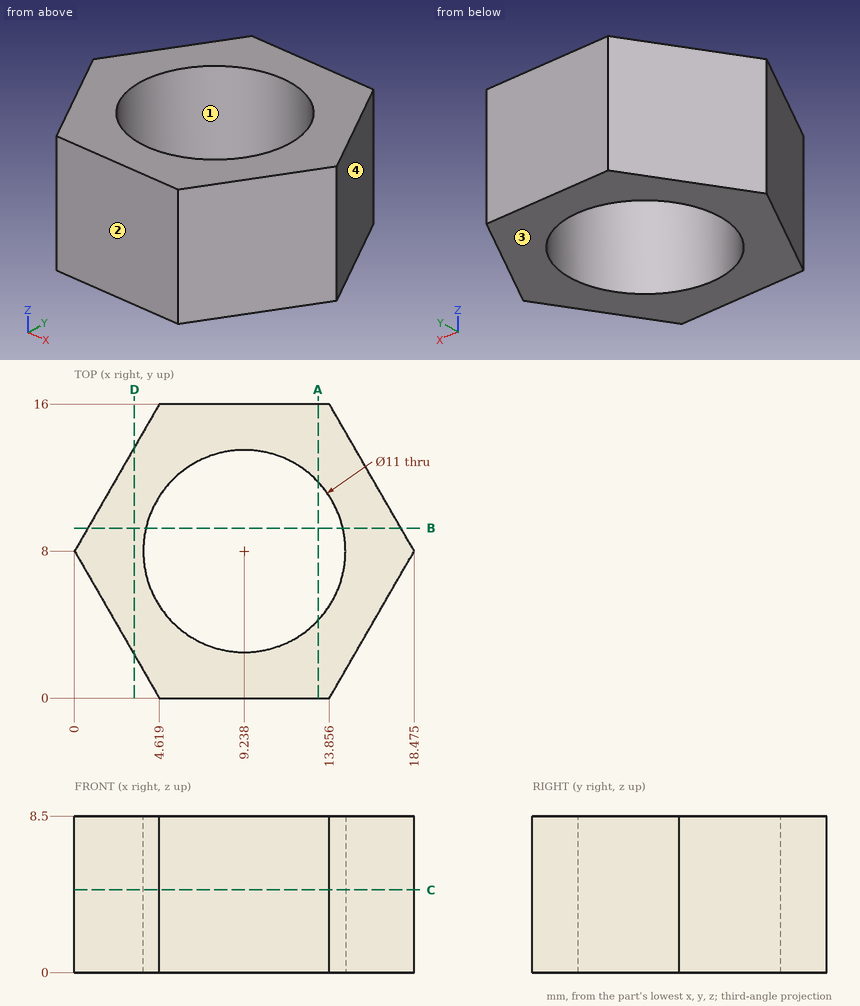
Can you work these out from the drawing? Everything is in mm from the part's minimum corner. Give positions to 0.01 mm unless a question says otherwise; leave off trailing zeros. Order: outer loops, then holes, each group sorted by start corner. A loop starts at its lowest first (then second) coordinate and runs counter-clockwise, first axis right, second up.
Item 1: If we mould it in two halves opening along Y, with no side actions, what happens to the marked faces 1, 2, 3 and 4? For each: pulls with the +Y half, pulls with the -Y half, needs draft (parallel to the pull), parting line crosses it, or undercut.
Item 2: If we section it at A-A, the plane x = 13.25: Write out the boundary of the cut face in (y, z).
Item 3: If we section it at B-B, the plane y = 9.25: Write out the boundary of the cut face in (x, z).
Item 4: I need wall thicknesses on line 1 (Y direction, x = 11.75, z = 6.5); line 2 (X direction, y = 11.25, z = 5.5) (1 decimal); line 3 (X direction, y = 11.75, z = 1) (1 decimal). Which ranges of each line are inside material? Lowest first, please.
Item 5: If we section it at D-D, the plane x = 3.25: Write out the boundary of the cut face in (y, z).
Item 6: If we section it at C-C, the plane z = 4.5: Write out the boundary of the cut face in (x, y) (1 decimal), plus the area to 3 significant figures.
Values:
1. face 1: undercut
1. face 2: pulls with the -Y half
1. face 3: needs draft
1. face 4: pulls with the +Y half
2. outline: (0, 0) - (4.24, 0) - (4.24, 8.5) - (0, 8.5) - close; (11.76, 0) - (16, 0) - (16, 8.5) - (11.76, 8.5) - close
3. outline: (0.72, 0) - (3.88, 0) - (3.88, 8.5) - (0.72, 8.5) - close; (14.59, 0) - (17.75, 0) - (17.75, 8.5) - (14.59, 8.5) - close
4. line 1: y = 0 to 3.11, 12.89 to 16
4. line 2: x = 1.9 to 4.8, 13.7 to 16.6
4. line 3: x = 2.2 to 5.2, 13.3 to 16.3
5. outline: (2.37, 0) - (13.63, 0) - (13.63, 8.5) - (2.37, 8.5) - close
6. outline: (0, 8) - (4.6, 0) - (13.9, 0) - (18.5, 8) - (13.9, 16) - (4.6, 16) - close; hole circle Ø11 at (9.2, 8)
6. area: 127 mm2
